Read the model definition and answer for the solid it produces. Units are mm, in the model's axes. A direction names the side the tool comes from. Coordinates: 2 decimals unless noted, no trailing zeros. Loops run counter-clockwise (first coordinate to the right, second up) from the corner with the lowest first, then second, coordinate; pieces in that order, holes last. Notation, with made-up numbers: (80, 24.5) -> (109, 24.5) arc R12 cw to (109, 44.5) -> close; hole circle Ø7 at (20.25, 54). An arc over 180 degrees is marked (long way). Answer as a JSON object with one key per item and string values. Group by question number.
Q1. This flat-tipped pin is pushed along its axis until it touches: P1, Ø3.5, axis at x = -13, y = -2.5, coming from the -Z side. Where does it stop, or does it pass through?
Q2. The part is cut by section C-C on y = -12.5. Write down the section's boundary in (x, z), and give its area (3 significant figures).
Q3. Determine the mould class of faces 6 (the cylindrical face through (7.6, 16, -3.8)), 7 (the flat face through (30, -17.5, -0.1)), 8 (the flat face through (-32.5, 0, 0)) for opening direction Y: released by +Y, released by -Y, zero draft, split by the parting line, or undercut.
Q4. For faces 1 (the flat face through (10, 8, 1)), 2 (the cylindrical face through (7.55, 1.75, 2.57)), 3 (the flat face through (0, 0, -8.5)), 4 (the cylindrical face through (7.6, 0, 6.3)), 5 (the flat face through (0, -20, 0)), determine the directions among +Z, -Z, +X, -X, +Y, -Y from which every point of the face is accessible in a straight line to the end or side of a thin tool.
Q5. The part is cut by section B-B on z = 6.25. Write down the section's boundary in (x, y).
Q6. Straight lines are drawn through the part: line 1 along Y through (x, z) = (-22.5, 3.75); line 2 along Y through (x, z) = (22.5, -4); line 3 along Y through (x, z) = (-12.5, -6). For each, find the intervals that lie inside material, in ascending order. Write a range as [from, to].
Q7. The part is cut by section D-D on x = -12.5. Write down the section's boundary in (y, z).
Q8. The part is cut by section A-A on x = 22.5. Write down the section's boundary in (y, z).
from build123d import *

# Parameters (mm, degrees)
SKETCH_1_W                   = 65
SKETCH_1_H                   = 40
EXTRUDE_1_DEPTH              = 8.5
HOLE_WIZARD_8_0_8_1_D        = 8
SKETCH_4_R                   = 6
CUT_EXTRUDE_1_DEPTH          = 9.5
HOLE_WIZARD_M4_1_D           = 4.5
HOLE_WIZARD_M4_1_CBORE_D     = 8
HOLE_WIZARD_M4_1_CBORE_DEPTH = 4.4
HOLE_WIZARD_6_0_6_1_D        = 6
CUT_EXTRUDE_2_DEPTH          = 9.5
CUT_EXTRUDE_3_DEPTH          = 42.776189391
CUT_EXTRUDE_START            = -4.4
CUT_EXTRUDE_4_DEPTH          = 4.4
CHAMFER_1_SIZE               = 5


with BuildPart() as part:
    # 草图1 → 凸台-拉伸1 (new, symmetric)
    with BuildSketch(Plane.XY):
        Rectangle(SKETCH_1_W, SKETCH_1_H)
    extrude(amount=EXTRUDE_1_DEPTH, both=True)

    # Ø8.0 (8) 直径孔1 (through all)
    with Locations(Plane.XY.offset(8.5)):
        with Locations((-22.5, 12.5), (-22.5, -12.5), (22.5, 0)):
            Hole(HOLE_WIZARD_8_0_8_1_D / 2)

    # 草图4 → 切除-拉伸1 (cut)
    with BuildSketch(Plane(origin=(0, 0, -8.5), x_dir=(-1, 0, 0), z_dir=(0, 0, -1))):
        with Locations((12.5, 0)):
            Circle(SKETCH_4_R)
    extrude(amount=-CUT_EXTRUDE_1_DEPTH, mode=Mode.SUBTRACT)

    # M4 六角凹头螺钉的柱形沉头孔1 (through all)
    with Locations(Plane.XY.offset(8.5)):
        with Locations((-12.5, 0)):
            CounterBoreHole(HOLE_WIZARD_M4_1_D / 2, HOLE_WIZARD_M4_1_CBORE_D / 2, HOLE_WIZARD_M4_1_CBORE_DEPTH)

    # Ø6.0 (6) 直径孔1 (through all)
    with Locations(Plane(origin=(0, 0, -8.5), x_dir=(-1, 0, 0), z_dir=(0, 0, -1))):
        with Locations((-7.5, -5)):
            Hole(HOLE_WIZARD_6_0_6_1_D / 2)

    # 草图9 → 切除-拉伸2 (cut)
    with BuildSketch(Plane(origin=(0, 0, -8.5), x_dir=(-1, 0, 0), z_dir=(0, 0, -1))):
        with BuildLine():
            Line((-11.5, 4), (-11.5, 12))
            ThreePointArc((-11.5, 12), (-7.5, 16), (-3.5, 12))
            Line((-3.5, 12), (-3.5, 4))
            ThreePointArc((-3.5, 4), (-7.5, 0), (-11.5, 4))
        make_face()
    extrude(amount=-CUT_EXTRUDE_2_DEPTH, mode=Mode.SUBTRACT)

    # 草图10 → 切除-拉伸3 (cut, through all)
    with BuildSketch(Plane.XY.offset(8.5)):
        with BuildLine():
            Line((5.25, 4), (5.25, 12))
            ThreePointArc((5.25, 12), (7.5, 14.25), (9.75, 12))
            Line((9.75, 12), (9.75, 4))
            ThreePointArc((9.75, 4), (7.5, 1.75), (5.25, 4))
        make_face()
    extrude(amount=-CUT_EXTRUDE_3_DEPTH, mode=Mode.SUBTRACT)

    # 草图11 → 切除-拉伸4 (cut)
    with BuildSketch(Plane.XY.offset(8.5).offset(CUT_EXTRUDE_START)):
        with BuildLine():
            Line((3.5, 4), (3.5, 12))
            ThreePointArc((3.5, 12), (7.5, 16), (11.5, 12))
            Line((11.5, 12), (11.5, 4))
            ThreePointArc((11.5, 4), (7.5, 0), (3.5, 4))
        make_face()
    extrude(amount=CUT_EXTRUDE_4_DEPTH, mode=Mode.SUBTRACT)

    # 倒角1
    chamfer_1_edges = [part.edges().sort_by_distance(p)[0] for p in [
        (32.5, -20, 0),
        (-32.5, -20, 0),
        (-32.5, 20, 0),
        (32.5, 20, 0),
    ]]
    chamfer(chamfer_1_edges, length=CHAMFER_1_SIZE)


solid = part.part
Final values:
{
 "1": {"P1": "stops at z = 1"},
 "2": {"outline": "(-32.5, -8.5) -> (-26.5, -8.5) -> (-26.5, 8.5) -> (-32.5, 8.5) -> close; (-18.5, -8.5) -> (32.5, -8.5) -> (32.5, 8.5) -> (-18.5, 8.5) -> close", "area": "969 mm2"},
 "3": {"face 6": "undercut", "face 7": "released by -Y", "face 8": "zero draft"},
 "4": {"face 1": "-Z", "face 2": "+Z, -Z", "face 3": "-Z, +X, -X, +Y, -Y", "face 4": "+Z", "face 5": "+Z, -Z, +X, -X, -Y"},
 "5": {"outline": "(-32.5, -15) -> (-27.5, -20) -> (27.5, -20) -> (32.5, -15) -> (32.5, 15) -> (27.5, 20) -> (-27.5, 20) -> (-32.5, 15) -> close; hole circle Ø8 at (-22.5, -12.5); hole circle Ø8 at (-22.5, 12.5); hole circle Ø8 at (-12.5, 0); hole (3.5, 4) arc R4 ccw to (11.5, 4) -> (11.5, 12) arc R4 ccw to (3.5, 12) -> close; hole circle Ø6 at (7.5, -5); hole circle Ø8 at (22.5, 0)"},
 "6": {"line 1": "y = [-20, -16.5], [-8.5, 8.5], [16.5, 20]", "line 2": "y = [-20, -4], [4, 20]", "line 3": "y = [-20, -6], [6, 20]"},
 "7": {"outline": "(-20, -8.5) -> (-6, -8.5) -> (-6, 1) -> (-2.25, 1) -> (-2.25, 4.1) -> (-4, 4.1) -> (-4, 8.5) -> (-20, 8.5) -> close; (2.25, 1) -> (6, 1) -> (6, -8.5) -> (20, -8.5) -> (20, 8.5) -> (4, 8.5) -> (4, 4.1) -> (2.25, 4.1) -> close"},
 "8": {"outline": "(-20, -8.5) -> (-4, -8.5) -> (-4, 8.5) -> (-20, 8.5) -> close; (4, -8.5) -> (20, -8.5) -> (20, 8.5) -> (4, 8.5) -> close"}
}
